Job drawing, mm, ordinate dimensions from the low corner. One solid piece. Give positions to 0.01 mm unless a question says otherwise; leave off trailing zeros. Order: outer loops, then holes, each group sorted by start corner. A loop starts at its lowest first (then second) coordinate and runs counter-clockwise, first axis right, second up. Notation, with made-up numbers: M 70,-31.75 L 81,-31.75 A31 ccw 81,5.25 Z; hole C 55,39 d3. An arc over 180 degrees is marked long. One line per question, with ' | ' between items.
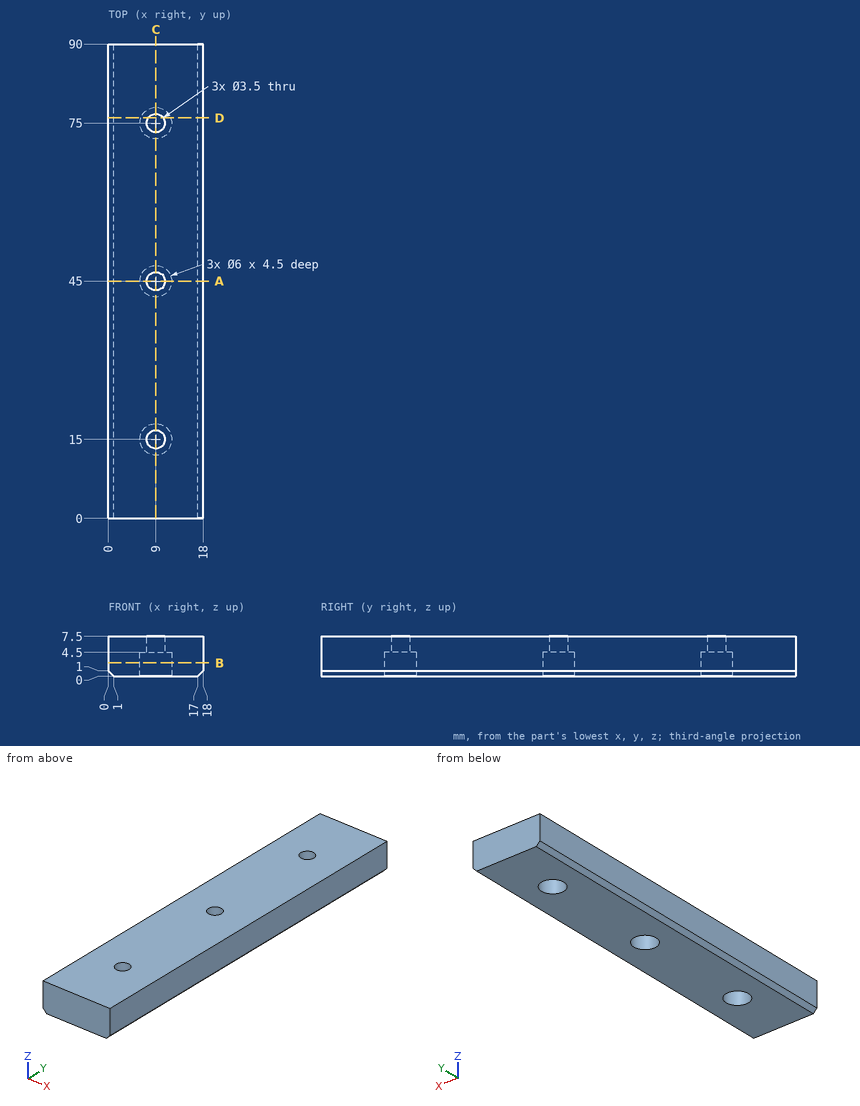
1. Slice it at A-A on y = 45. Give the cut face in (x, z), then the cut area to 3 significant figures.
Worked out:
outline: M 0,1 L 1,0 L 6,0 L 6,4.5 L 7.25,4.5 L 7.25,7.5 L 0,7.5 Z; M 10.75,4.5 L 12,4.5 L 12,0 L 17,0 L 18,1 L 18,7.5 L 10.75,7.5 Z | area: 96.5 mm2
2. Slice it at D-D on y = 76. Give the cut face in (x, z), then the cut area to 3 significant figures.
Worked out:
outline: M 0,1 L 1,0 L 6.17,0 L 6.17,4.5 L 7.56,4.5 L 7.56,7.5 L 0,7.5 Z; M 10.44,4.5 L 11.83,4.5 L 11.83,0 L 17,0 L 18,1 L 18,7.5 L 10.44,7.5 Z | area: 99.9 mm2
3. Slice it at C-C on x = 9. Give the cut face in (y, z), then the cut area to 4 significant figures.
Worked out:
outline: M 0,0 L 12,0 L 12,4.5 L 13.25,4.5 L 13.25,7.5 L 0,7.5 Z; M 16.75,4.5 L 18,4.5 L 18,0 L 42,0 L 42,4.5 L 43.25,4.5 L 43.25,7.5 L 16.75,7.5 Z; M 46.75,4.5 L 48,4.5 L 48,0 L 72,0 L 72,4.5 L 73.25,4.5 L 73.25,7.5 L 46.75,7.5 Z; M 76.75,4.5 L 78,4.5 L 78,0 L 90,0 L 90,7.5 L 76.75,7.5 Z | area: 562.5 mm2
4. Slice it at B-B on z = 2.5. Give the cut face in (x, y), then the cut area to 3 significant figures.
Worked out:
outline: M 0,0 L 18,0 L 18,90 L 0,90 Z; hole C 9,15 d6; hole C 9,45 d6; hole C 9,75 d6 | area: 1,540 mm2
5. Drop a flat-ended pin along its axis: pin 1 (1.8 mm diameter, centred on x = 9, y = 44.5, fed in from -Z). Give the stop position or say it passes through.
Worked out:
pin 1: passes through
6. Probe L1, parallel to Y at x = 9, z = 2.4; L2, parallel to Z at x = 8.75, y = 72.5; L3, parallel to Y at x = 10, z = 6.25. List the from-to ranges inside material, lowest first. Write a range as from..to.
Worked out:
L1: y = 0..12, 18..42, 48..72, 78..90 | L2: z = 4.5..7.5 | L3: y = 0..13.56, 16.44..43.56, 46.44..73.56, 76.44..90
